from build123d import *

# Parameters (mm, degrees)
SKETCH1_R           = 23
BOSS_EXTRUDE1_DEPTH = 420
CHAMFER1_SIZE       = 5
CHAMFER1_SIZE2      = 1.339745962
SKETCH2_R           = 12.5
BOSS_EXTRUDE2_DEPTH = 80
CHAMFER2_SIZE       = 2


with BuildPart() as part:
    # Sketch1 → Boss-Extrude1 (new body)
    with BuildSketch(Plane.XY):
        Circle(SKETCH1_R)
    extrude(amount=BOSS_EXTRUDE1_DEPTH)

    # Chamfer1
    chamfer1_edges = [part.edges().sort_by_distance(p)[0] for p in [
        (-23, 0, 420),
    ]]
    chamfer1_side = [part.faces().sort_by_distance(p)[0] for p in [
        (-23, 0, 210),
    ]]
    chamfer(chamfer1_edges, length=CHAMFER1_SIZE, length2=CHAMFER1_SIZE2, reference=chamfer1_side[0])

    # Sketch2 → Boss-Extrude2 (add)
    with BuildSketch(Plane(origin=(0, 0, 0), x_dir=(-1, 0, 0), z_dir=(0, 0, -1))):
        with Locations(Location((0, 0, 0), (0, 0, 180))):
            Circle(SKETCH2_R)
    extrude(amount=BOSS_EXTRUDE2_DEPTH)

    # Chamfer2
    chamfer2_edges = [part.edges().sort_by_distance(p)[0] for p in [
        (-23, 0, 0),
        (-12.5, 0, -80),
    ]]
    chamfer(chamfer2_edges, length=CHAMFER2_SIZE)


solid = part.part
Part model, mm, in its own coordinate system. Coordinates: 2 decimals unless noted, no trailing zeros. Loops run counter-clockwise (first coordinate to the right, second up) from the corner with the lowest first, then second, coordinate; pieces in that order, holes last. Notation, with made-up numbers: (60.25, 38) -> (72.25, 38) arc R24 cw to (72.25, 69) -> close; hole circle Ø9 at (11, -2.5). An arc over 180 degrees is marked (long way). Use a Markdown table: item, result. Add a question column.
Item 1: Pull direction Z, two halves, no side cores. Call faces 1 (the cylindrical face through (11.923, -3.755, -38.454)), 2 (the flat face through (9, -9, 0)), 3 (the conical face through (-4.7, -21.2, 419.8)): +Z half, -Z half, draft (parallel to the pull), parting line (faces both ways), or undercut.
Item 2: Band-saw the part on C-C on z = 106.5. Write the cut outline in (x, y), plus the area to 3 significant figures.
Item 3: Probe probe 1 along Y at (x, z) = (-7.5, 134.5); probe 2 along Y at (x, z) = (-1, 296); probe 3 along Z at (x, y) = (7, 14.5). List the from-to ranges inside material, lowest first.
Item 4: Flat gauge pins, fed straight in: P1, Ø5, axis at y = 7.5, z = 259.5, coming from the -X side; P2, Ø1, axis at x = -3, z = 191, coming from the +Y side; P3, Ø2, axis at y = 3.5, z = 359, coming from the -X side. Where does each tip first touch, or does it go through?
Item 5: Band-saw the part on A-A on x = 0. Write the cut outline in (y, z).
Geometry says:
| question | item | result |
|---|---|---|
| 1 | face 1 | draft |
| 1 | face 2 | -Z half |
| 1 | face 3 | +Z half |
| 2 | outline | circle Ø46 at (0, 0) |
| 2 | area | 1,660 mm² |
| 3 | probe 1 | -21.74 to 21.74 |
| 3 | probe 2 | -22.98 to 22.98 |
| 3 | probe 3 | 0 to 420 |
| 4 | P1 | x = -22.45 |
| 4 | P2 | y = 22.86 |
| 4 | P3 | x = -22.86 |
| 5 | outline | (-23, 2) -> (-21, 0) -> (-12.5, 0) -> (-12.5, -78) -> (-10.5, -80) -> (10.5, -80) -> (12.5, -78) -> (12.5, 0) -> (21, 0) -> (23, 2) -> (23, 415) -> (21.66, 420) -> (-21.66, 420) -> (-23, 415) -> close |
